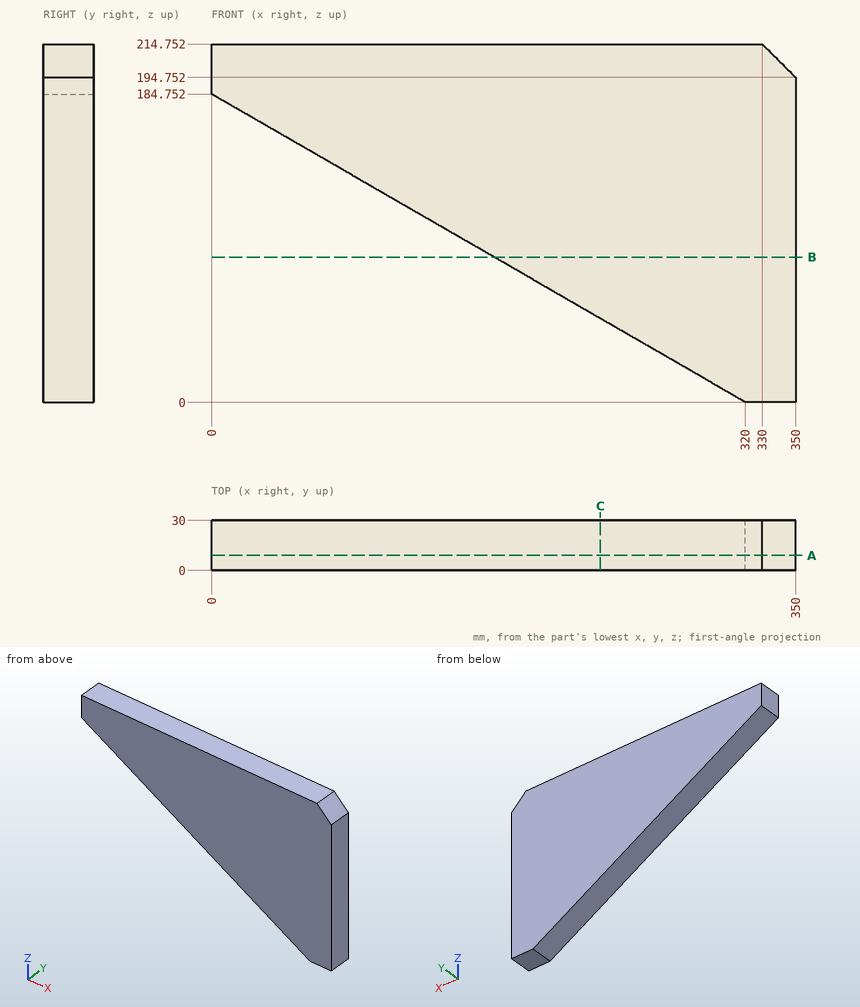
Here's the drawing with two shaded views (mm, measured from the low corner). I have some questions. Coordinates: 2 decimals unless noted, no trailing zeros. Write each loop counter-clockwise with the first axis right and the second up, starting at its lowest first coordinate (ties: lowest second). Pieces come first, ordered by that corner, then holes. Notation, with made-up numbers: (-4, 6) - (29, 6) arc R24 cw to (29, 38) - close; hole circle Ø2 at (-5, 51.25). An arc over 180 degrees is marked (long way). Return JSON: item names as keys, results as strings.
Q1. Please list where these lines run through material, in increasing order: L1, parallel to X at y = 5.25, z = 69.5; L2, parallel to X at y = 20.5, z = 95 (1 decimal); L3, parallel to Z at x = 333, y = 17.75. Write a range as from..to.
Computed values:
{"L1": "x = 199.62..350", "L2": "x = 155.5..350", "L3": "z = 0..211.75"}
Q2. If we section it at B-B (z = 87): Please give me the cut outline in (x, y).
Computed values:
{"outline": "(169.31, 0) - (350, 0) - (350, 30) - (169.31, 30) - close"}
Q3. I'm going to push flat-ended pins straight in: pin 1 Ø1.5 at (x, y) = (217.5, 16.5) entering from -Z; pin 2 Ø6 at (y, z) = (9.5, 103) entering from -X; pin 3 Ø3 at (x, y) = (165.5, 14) entering from -Z. Where does each tip first touch, or does it pass through?
Computed values:
{"pin 1": "stops at z = 58.75", "pin 2": "stops at x = 136.4", "pin 3": "stops at z = 88.33"}
Q4. If we section it at A-A (y = 9): Please give me the cut outline in (x, z).
Computed values:
{"outline": "(0, 184.75) - (320, 0) - (350, 0) - (350, 194.75) - (330, 214.75) - (0, 214.75) - close"}
Q5. If we section it at C-C (x = 233): Please give me the cut outline in (y, z), then the cut area to 3 significant figures.
Computed values:
{"outline": "(0, 50.23) - (30, 50.23) - (30, 214.75) - (0, 214.75) - close", "area": "4,940 mm2"}
